from build123d import *

# Parameters (mm, degrees)
BASE_DEPTH = 1200


with BuildPart() as part:
    # Sketch1 → Base (new body)
    with BuildSketch(Plane.YZ):
        with BuildLine():
            Line((0, 50), (0, 0))
            Line((0, 0), (50, 0))
            Line((50, 0), (50, 2))
            ThreePointArc((50, 2), (49.707106781, 2.707106781), (49, 3))
            Line((49, 3), (8.5, 3))
            ThreePointArc((8.5, 3), (4.610912703, 4.610912703), (3, 8.5))
            Line((3, 8.5), (3, 49))
            ThreePointArc((3, 49), (2.707106781, 49.707106781), (2, 50))
            Line((2, 50), (0, 50))
        make_face()
    extrude(amount=BASE_DEPTH)


solid = part.part
The model under review builds one solid part; all positions refer to its coordinate system, in mm. A direction names the side the tool comes from. Round coordinates to 2 decimals unless told otherwise and drop trailing zeros. Order: outer loops, then holes, each group sorted by start corner. A loop starts at its lowest first (then second) coordinate and runs counter-clockwise, first axis right, second up. Notation, with made-up numbers: (61, -6) -> (96, -6) arc R20 cw to (96, 7) -> close; hole circle Ø10 at (51.5, 4.5). An arc over 180 degrees is marked (long way). Write item = value, one per line. Start each with the question number.
Item 1: For faces 1 (the face through (592, 29, 3)), 2 (the face through (0, 2.7, 14)), list the 3-axis set-ups (+Z, -Z, +X, -X, +Y, -Y) from which the entire face can be reached by the end or side of a thin tool; tool diameter is ignored.
Item 2: Clearance check with flat-ended pins moving along their axes: pin 1 Ø1.5 at (x, z) = (721, 23.5) entering from +Y; pin 2 Ø20 at (x, y) = (820.5, 19.5) entering from +Z. State where each tip first meets the part, or that it passes through.
Item 3: Consider section A-A on x = 775.5. Write out the cut boundary in (y, z), plus the area to 3 significant figures.
Item 4: For line 1 along Z through (x, y) = (343, 21); line 2 along Y through (x, z) = (475.5, 7.5), list the stretches that pass through material, from the lowest coordinate up.
Item 5: Consider section B-B on y = 25. Write out the cut boundary in (x, z).
Conclusion:
q1.face_1 = +Z, +X, -X, +Y
q1.face_2 = +Z, -Z, -X, +Y, -Y
q2.pin_1 = 3
q2.pin_2 = 3
q3.outline = (0, 0) -> (50, 0) -> (50, 2) arc R1 ccw to (49, 3) -> (8.5, 3) arc R5.5 cw to (3, 8.5) -> (3, 49) arc R1 ccw to (2, 50) -> (0, 50) -> close
q3.area = 297 mm2
q4.line_1 = 0 to 3
q4.line_2 = 0 to 3.09
q5.outline = (0, 0) -> (1200, 0) -> (1200, 3) -> (0, 3) -> close
